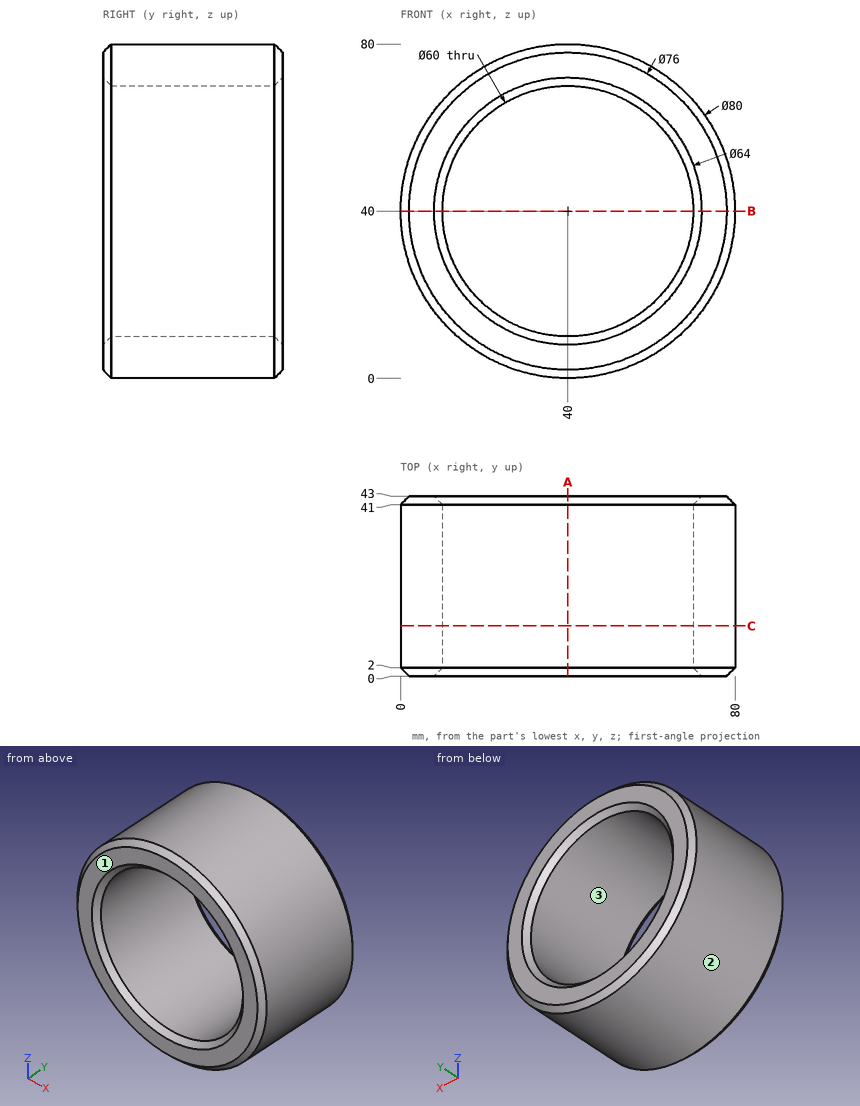
Geometry: see drawing. Coordinates: mm, zero at the bounding-box minimum. Give positions to 0.01 mm unless a question says otherwise; leave off trailing zeros. Order: outer loops, then holes, each group sorted by start corner. A loop starts at its lowest first (then second) coordinate and runs counter-clockwise, first axis right, second up. Notation, with made-up numbers: M 7,-30.5 L 24,-30.5 A22 ccw 24,7.5 Z; hole C -12,40 d10. An arc over 180 degrees is marked long. Answer as a JSON object with one key per item and string values.
1. Cut plane C-C, the plane y = 12. Output: boundary loops of the cut face in (x, z), and give its area (3 significant figures).
Result sheet:
{"outline": "C 40,40 d80; hole C 40,40 d60", "area": "2,200 mm²"}
2. Cut plane A-A, the plane x = 40. Output: boundary loops of the cut face in (y, z).
Result sheet:
{"outline": "M 0,2 L 2,0 L 41,0 L 43,2 L 43,8 L 41,10 L 2,10 L 0,8 Z; M 0,72 L 2,70 L 41,70 L 43,72 L 43,78 L 41,80 L 2,80 L 0,78 Z"}
3. Pull-direction query (X, two-part tool) for the marked faces 1, 2 and 3; classes: +X half, -X half, draft (parallel to the pull), parting line (faces both ways), or undercut.
Result sheet:
{"face 1": "draft", "face 2": "parting line", "face 3": "undercut"}
4. First-contact query: P1, Ø2, axis at x = 68.5, y = 13, coming from the -Z side; P2, Ø2, axis at y = 38, z = 21, coming from the +X side; P3, Ø12, axis at y = 34.5, z = 38.5, coming from the +X side. Flat tips, straight axial feed; report the tip coordinate or a pass-through.
Result sheet:
{"P1": "z = 10.95", "P2": "x = 75.72", "P3": "x = 80"}
5. Ray query, line 1 (X direction, y = 33, z = 40); line 2 (Z direction, x = 67, y = 7.5); line 3 (Z direction, x = 44, y = 41). Return the intervals inside material, ascending. Write a range as [from, to].
Result sheet:
{"line 1": "[0, 10], [70, 80]", "line 2": "[10.49, 26.92], [53.08, 69.51]", "line 3": "[0.2, 10.27], [69.73, 79.8]"}
6. Cut plane B-B, the plane z = 40. Output: boundary loops of the cut face in (x, y), and give its area (3 significant figures).
Result sheet:
{"outline": "M 0,2 L 2,0 L 8,0 L 10,2 L 10,41 L 8,43 L 2,43 L 0,41 Z; M 70,2 L 72,0 L 78,0 L 80,2 L 80,41 L 78,43 L 72,43 L 70,41 Z", "area": "844 mm²"}
